Source: CAD feature listing. Evaluate the final solid. Frame: model axes, mm. Coordinates: 2 decimals unless noted, no trailing zeros. Write each loop counter-clockwise with the first axis right and the second up, starting at its lowest first coordinate (ties: lowest second). Pieces come first, ordered by that corner, then holes. Notation, with made-up numbers: M 78.25,67 L 129.25,67 A18 cw 129.25,89 Z; hole C -3,67.25 d7. An arc over 180 degrees is marked long. One line per item, written item: value. Start each with the question number.
Item 1: Mould query, pull axis X, two halves, no side actions, for faces 1 (the cylindrical face through (-6.777, 1.802, 4.93)), 2 (the flat face through (40.1, 42.4, 4.9)), 3 (the flat face through (-1, 1, 0)). Classes: released by +X, released by -X, zero draft, split by the parting line, or undercut.
Item 2: Cut plane B-B, the plane y = 0. Output: boundary loops of the cut face in (x, z), then the cut area to 3 significant figures.
Item 3: Cut plane C-C, the plane z = 3. Output: boundary loops of the cut face in (x, y).
Item 4: Cut plane A-A, the plane x = -12.5. Output: boundary loops of the cut face in (y, z), then the cut area to 3 significant figures.
Item 5: Ray query, L1, parallel to Y at x = -12.5, z = 4; L2, parallel to X at y = 2, z = 8.75; L3, parallel to Y at x = 30.5, z = 2.5. Return the intervals inside material, ascending. Write a range as from..to.
Item 6: Cut plane D-D, the plane x = 30.5. Output: boundary loops of the cut face in (y, z).
Item 7: Pin query (flat end, axial travel): P1, Ø11, axis at x = 30.5, y = 0, coming from the -Z side (3 decimals). Return the tip coordinate at first contact, or that it passes through.
```python
from build123d import *

# Parameters (mm, degrees)
SKETCH_1_R      = 6
SKETCH_1_R_2    = 9
EXTRUDE_1_DEPTH = 10


with BuildPart() as part:
    # 草图1 → 凸台-拉伸1 (new body)
    with BuildSketch(Plane.XY):
        Polygon((47.5, 35), (32.5, 50), (-47.5, 50), (-47.5, -50), (32.5, -50), (47.5, -35), align=None)
        with Locations((-12.5, 0)):
            Circle(SKETCH_1_R, mode=Mode.SUBTRACT)
        with Locations((30.5, 0)):
            Circle(SKETCH_1_R_2, mode=Mode.SUBTRACT)
    extrude(amount=EXTRUDE_1_DEPTH)


solid = part.part
```
From the geometry:
1. face 1: undercut
1. face 2: released by +X
1. face 3: zero draft
2. outline: M -47.5,0 L -18.5,0 L -18.5,10 L -47.5,10 Z; M -6.5,0 L 21.5,0 L 21.5,10 L -6.5,10 Z; M 39.5,0 L 47.5,0 L 47.5,10 L 39.5,10 Z
2. area: 650 mm²
3. outline: M -47.5,-50 L 32.5,-50 L 47.5,-35 L 47.5,35 L 32.5,50 L -47.5,50 Z; hole C -12.5,0 d12; hole C 30.5,0 d18
4. outline: M -50,0 L -6,0 L -6,10 L -50,10 Z; M 6,0 L 50,0 L 50,10 L 6,10 Z
4. area: 880 mm²
5. L1: y = -50..-6, 6..50
5. L2: x = -47.5..-18.16, -6.84..21.73, 39.27..47.5
5. L3: y = -50..-9, 9..50
6. outline: M -50,0 L -9,0 L -9,10 L -50,10 Z; M 9,0 L 50,0 L 50,10 L 9,10 Z
7. P1: passes through
